Verification items for the finished model (mm, model axes). Give positions to 0.01 mm unless a question says otherwise; leave off trailing zeros. Order: outer loops, then holes, each group sorted by start corner. A loop starts at its lowest first (then second) coordinate and runs counter-clockwise, first axis right, second up.
from build123d import *

# Parameters (mm, degrees)
SKETCH_1_R          = 16.85
SKETCH_1_R_2        = 13.95
EXTRUDE_1_DEPTH     = 1100
SKETCH_2_R          = 3
CUT_EXTRUDE_1_DEPTH = 16.85


with BuildPart() as part:
    # 草图1 → 凸台-拉伸1 (new body)
    with BuildSketch(Plane.XY):
        Circle(SKETCH_1_R)
        Circle(SKETCH_1_R_2, mode=Mode.SUBTRACT)
    extrude(amount=EXTRUDE_1_DEPTH)

    # 草图2 → 切除-拉伸1 (cut, symmetric)
    with BuildSketch(Plane(origin=(0, 0, 0), x_dir=(1, 0, 0), z_dir=(0, 1, 0))):
        with Locations(Location((0, -15, 0), (0, 0, 270))):
            Circle(SKETCH_2_R)
        with Locations(Location((0, -1085, 0), (0, 0, 270))):
            Circle(SKETCH_2_R)
    extrude(amount=CUT_EXTRUDE_1_DEPTH, both=True, mode=Mode.SUBTRACT)


solid = part.part
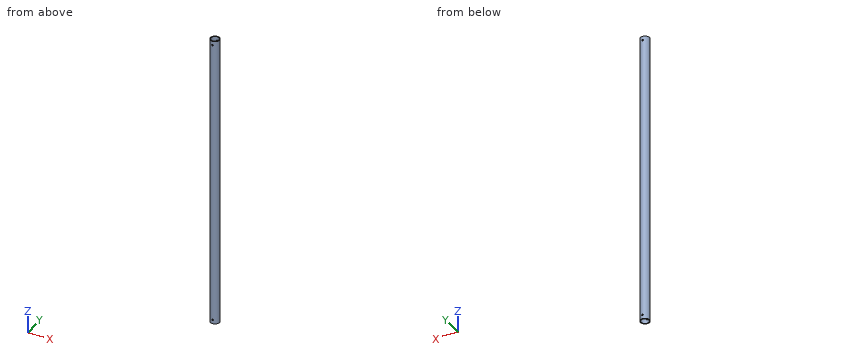
(1) Go/stop test with flat-tipped pins: pin 1 (4 mm diameter, centred on y = -2, z = 159.5, fed in from -X); pin 2 (6 mm diameter, centred on x = 7.5, z = 886, fed in from +Y). Record where each tip stops, or that it passes through.
Solved:
pin 1: stops at x = -16.85
pin 2: stops at y = 16.24
(2) Scan lines: line 1 (Z direction, x = 0, y = 15); line 2 (X direction, y = -1.5, z = 932.5); line 3 (Y direction, x = 0, z = 89). Record each from-to range of solid material in increasing order.
Solved:
line 1: z = 0 to 12, 18 to 1082, 1088 to 1100
line 2: x = -16.78 to -13.87, 13.87 to 16.78
line 3: y = -16.85 to -13.95, 13.95 to 16.85
(3) Section check A-A, the plane y = 0. Enter the section's corners in (x, z), then the cut area to 3 significant figures.
Solved:
outline: (-16.85, 0) - (-13.95, 0) - (-13.95, 1100) - (-16.85, 1100) - close; (13.95, 0) - (16.85, 0) - (16.85, 1100) - (13.95, 1100) - close
area: 6,380 mm2
(4) Section check B-B, the plane z = 149. Enter the section's corners in (x, y), then the cut area to 3 significant figures.
Solved:
outline: circle Ø33.7 at (0, 0); hole circle Ø27.9 at (0, 0)
area: 281 mm2
